For this review, use the dimensioned drawing (mm, ordinates from the lowest corner) and the shaded views. Coordinates: 2 decimals unless noted, no trailing zeros. Order: outer loops, then holes, each group sorted by start corner. A loop starts at its lowest first (then second) coordinate and runs counter-clockwise, first axis right, second up. Notation, with made-up numbers: M -27,-29.75 L 21,-29.75 A24 ccw 21,-6.75 Z; hole C 87,48.25 d6. An arc over 180 degrees is marked long. One line per item, written item: value.
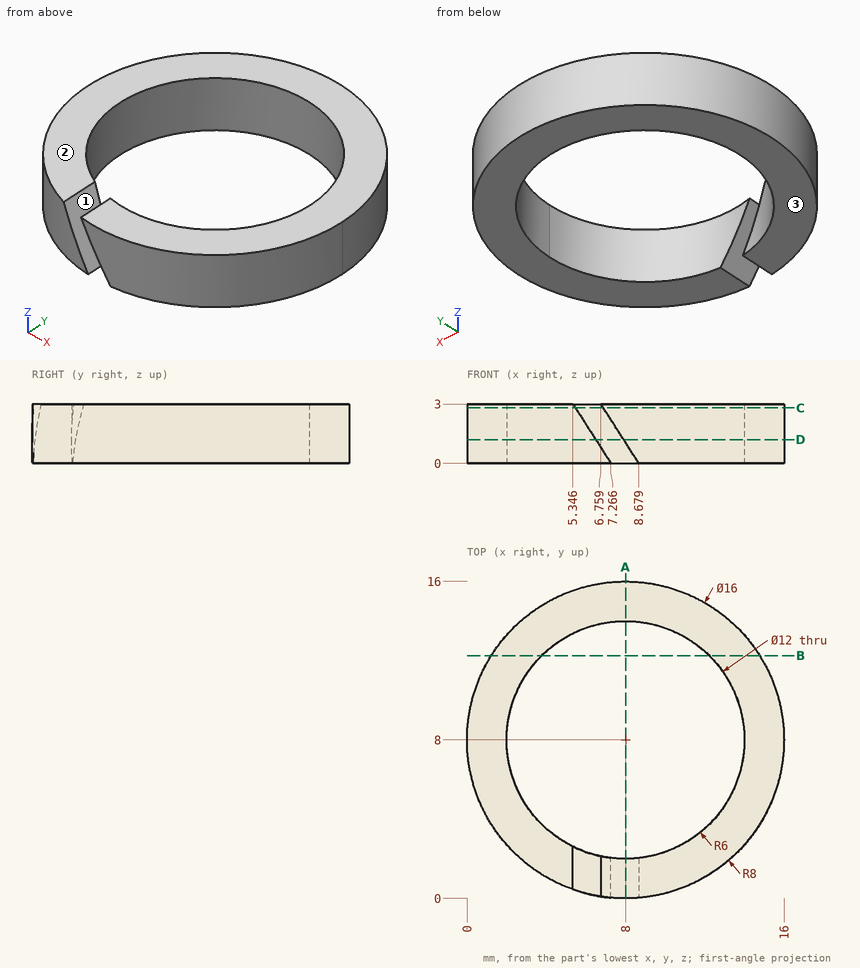
(1) We need section C-C, the plane z = 2.8. State the section outline as (x, y) points.
Geometry results:
outline: M 5.47,0.41 L 5.47,2.56 A6 cw long 6.89,2.1 L 6.89,0.08 A8 ccw long Z
(2) Mouldability with a two-part tool opening along Z and no side actions: class the marked faces 1, 2 and 3 as +Z half, -Z half, draft (parallel to the pull), parting line (faces both ways), or undercut.
Geometry results:
face 1: undercut
face 2: +Z half
face 3: -Z half
(3) Insertion check: pin 1 Ø1 at (x, z) = (10, 2.5) entering from -Y; pin 2 Ø6 at (x, y) = (1.5, 13) entering from +Z; pin 3 Ø1.5 at (y, z) = (11, 1.5) entering from +X. Each pin has a flat end and moves straight along its axis. Give the tip position at first contact, or say it passes through.
Geometry results:
pin 1: stops at y = 0.14
pin 2: stops at z = 3
pin 3: stops at x = 15.68
(4) We need section B-B, the plane y = 12.25. State the section outline as (x, z) points (1 decimal).
Geometry results:
outline: M 1.2,0 L 3.8,0 L 3.8,3 L 1.2,3 Z; M 12.2,0 L 14.8,0 L 14.8,3 L 12.2,3 Z
(5) We need section A-A, the plane x = 8. State the section outline as (y, z) points.
Geometry results:
outline: M 0,1.06 L 2,1.06 L 2,3 L 0,3 Z; M 14,0 L 16,0 L 16,3 L 14,3 Z
(6) We need section D-D, the plane z = 1.2. State the section outline as (x, y) points.
Geometry results:
outline: M 6.5,0.14 L 6.5,2.19 A6 cw long 7.91,2 L 7.91,0 A8 ccw long Z
(7) For L1, parallel to X at y = 8, z = 1.8; L2, parallel to Y at x = 11.75, z = 1.55 (1 decimal), list the stretches that pass through material, from the lowest coordinate up.
Geometry results:
L1: x = 0 to 2, 14 to 16
L2: y = 0.9 to 3.3, 12.7 to 15.1
